```python
from build123d import *


with BuildPart() as part:
    # 草图1 → 旋转1 (revolve)
    with BuildSketch(Plane(origin=(0, 0, 0), x_dir=(-1, 0, 0), z_dir=(0, 0, -1)), mode=Mode.PRIVATE) as revolve_1_sk:
        Polygon((-5, -19), (0, -19), (0, 19), (-5, 19), (-5, 17), (-4.5, 17), (-4.5, 15.8), (-5, 15.8), (-5, -15.8), (-4.5, -15.8), (-4.5, -17), (-5, -17), align=None)
    revolve(revolve_1_sk.sketch.rotate(Axis((0, -19, 0), (0, 1, 0)), 270), axis=Axis((0, -19, 0), (0, 1, 0)))


solid = part.part
```
Part model, mm, in its own coordinate system. A direction names the side the tool comes from. Give positions to 0.01 mm unless a question says otherwise; leave off trailing zeros. Write each loop counter-clockwise with the first axis right and the second up, starting at its lowest first coordinate (ties: lowest second). Pieces come first, ordered by that corner, then holes. Notation, with made-up numbers: M 8.5,76 L 14.5,76 A21 ccw 14.5,103 Z; hole C 10,54 d5. An arc over 180 degrees is marked long. Use CSV: the item, a comma, the result in double quotes.
Item 1: Pin check, flat tips, straight feed: P1, Ø3, axis at y = -14.5, z = -2, coming from the -X side; P2, Ø2, axis at x = 2.5, y = 13, coming from the -Z side; P3, Ø5, axis at x = 3, y = 6, coming from the -Z side. Stop position of each tip, or through.
Taken from the geometry:
P1,"stops at x = -4.97"
P2,"stops at z = -4.77"
P3,"stops at z = -4.97"
Item 2: Slice it at C-C on y = -5. Write the cut outline in (x, z), plus the area to 3 significant figures.
Taken from the geometry:
outline,"C 0,0 d10"
area,"78.5 mm²"
Item 3: Which spindle directions (+Z, -Z, +X, -X, +Y, -Y) get a long thin tool onto all of the face, cutting with end or side? Do faces 1 (the face through (-4.88, -0.22, -1.08)), 2 (the face through (1.352, -16.408, 4.292)). Say none if no direction does.
Taken from the geometry:
face 1,"+Y, -Y"
face 2,"none"
Item 4: Slice it at B-B on z = -2.5. Write the cut outline in (x, y).
Taken from the geometry:
outline,"M -4.33,-19 L 4.33,-19 L 4.33,-17 L 3.74,-17 L 3.74,-15.8 L 4.33,-15.8 L 4.33,15.8 L 3.74,15.8 L 3.74,17 L 4.33,17 L 4.33,19 L -4.33,19 L -4.33,17 L -3.74,17 L -3.74,15.8 L -4.33,15.8 L -4.33,-15.8 L -3.74,-15.8 L -3.74,-17 L -4.33,-17 Z"
Item 5: Drill centre lines: probe 1 along Y at (x, z) = (-2.5, 4); probe 2 along Z at (x, y) = (-4, 2); probe 3 along Z at (x, y) = (-2, 2). Where is each one in solid material? Low to high.
Taken from the geometry:
probe 1,"y = -19 to -17, -15.8 to 15.8, 17 to 19"
probe 2,"z = -3 to 3"
probe 3,"z = -4.58 to 4.58"
Item 6: Slice it at A-A on x = -3. Write the cut outline in (y, z).
Taken from the geometry:
outline,"M -19,-4 L -17,-4 L -17,-3.35 L -15.8,-3.35 L -15.8,-4 L 15.8,-4 L 15.8,-3.35 L 17,-3.35 L 17,-4 L 19,-4 L 19,4 L 17,4 L 17,3.35 L 15.8,3.35 L 15.8,4 L -15.8,4 L -15.8,3.35 L -17,3.35 L -17,4 L -19,4 Z"
Item 7: Pull direction Y, two halves, no side cores. Call faces 3 (the face through (1.352, 16.392, 4.292)), 4 (the face through (-4.88, -18.01, -1.08)), 5 (the face through (0, 19, 0)): +Y half, -Y half, draft (parallel to the pull), parting line (faces both ways), or undercut.
Taken from the geometry:
face 3,"undercut"
face 4,"draft"
face 5,"+Y half"
